```python
from build123d import *

# Parameters (mm, degrees)
SKETCH_1_W          = 200
SKETCH_1_H          = 140
EXTRUDE_1_DEPTH     = 1.5
SKETCH_2_R          = 4
CUT_EXTRUDE_1_DEPTH = 11.5


with BuildPart() as part:
    # 草图1 → 凸台-拉伸1 (new, symmetric)
    with BuildSketch(Plane.XY):
        Rectangle(SKETCH_1_W, SKETCH_1_H)
    extrude(amount=EXTRUDE_1_DEPTH, both=True)

    # 草图2 → 切除-拉伸1 (cut, symmetric)
    with BuildSketch(Plane.XY):
        with Locations((60, 0)):
            Circle(SKETCH_2_R)
    extrude(amount=CUT_EXTRUDE_1_DEPTH, both=True, mode=Mode.SUBTRACT)


solid = part.part
```
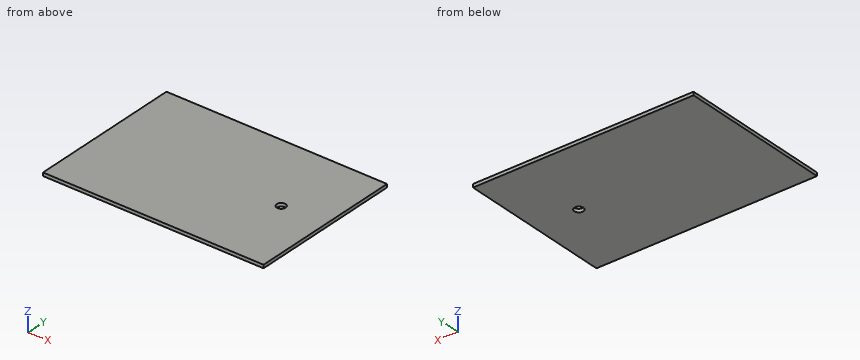
Verification items for the finished model (mm, model axes). Give positions to 0.01 mm unless a question says otherwise; leave off trailing zeros. Loops run counter-clockwise (first coordinate to the right, second up) from the corner with the lowest first, then second, coordinate; pieces in that order, holes last.
1. Section check B-B, the plane y = 0. Enter the section's corners in (x, z).
2. Go/stop test with a flat-tipped pin: pin 1 Ø13 at (x, y) = (60, 0) entering from -Z. Record where the tip stops, or that it passes through.
3. Section check A-A, the plane x = 60. Enter the section's corners in (y, z).
4. Thickness scan on line 1 (Y direction, x = 60, z = 0.1); line 2 (X direction, y = -2.5, z = -0.7); line 3 (X direction, y = -1, z = -0.05). Record the ranges inside material, lowest first.
Geometry says:
1. outline: (-100, -1.5) - (56, -1.5) - (56, 1.5) - (-100, 1.5) - close; (64, -1.5) - (100, -1.5) - (100, 1.5) - (64, 1.5) - close
2. pin 1: stops at z = -1.5
3. outline: (-70, -1.5) - (-4, -1.5) - (-4, 1.5) - (-70, 1.5) - close; (4, -1.5) - (70, -1.5) - (70, 1.5) - (4, 1.5) - close
4. line 1: y = -70 to -4, 4 to 70
4. line 2: x = -100 to 56.88, 63.12 to 100
4. line 3: x = -100 to 56.13, 63.87 to 100
